```python
from build123d import *

# Parameters (mm, degrees)
SKETCH1_W          = 50
SKETCH1_H          = 70
M16_TAPPED_HOLE1_D = 14
CIRPATTERN1_COUNT  = 4


with BuildPart() as part:
    # Sketch1 → Revolve1 (revolve)
    with BuildSketch(Plane.XY, mode=Mode.PRIVATE) as revolve1_sk:
        with Locations((0, 65)):
            Rectangle(SKETCH1_W, SKETCH1_H)
    revolve(revolve1_sk.sketch.rotate(Axis((71.901236476, 0, 0), (-1, 0, 0)), 90), axis=Axis((71.901236476, 0, 0), (-1, 0, 0)))

    # M16 Tapped Hole1 (through all)
    with Locations(Plane(origin=(-25, 0, -75), x_dir=(0, 0, -1), z_dir=(-1, 0, 0))):
        with Locations((0, 0)):
            m16_tapped_hole1 = Hole(M16_TAPPED_HOLE1_D / 2)

    # CirPattern1: M16 Tapped Hole1 ×4 about axis
    cirpattern1_axis = Axis((0, 0, 0), (1, 0, 0))
    for i in range(1, CIRPATTERN1_COUNT):
        add(m16_tapped_hole1.rotate(cirpattern1_axis, i * 360 / CIRPATTERN1_COUNT), mode=Mode.SUBTRACT)


solid = part.part
```
Can you work these out from the model? Positions are in its coordinate system, mm. Give positions to 0.01 mm unless a question says otherwise; leave off trailing zeros. Order: outer loops, then holes, each group sorted by start corner. A loop starts at its lowest first (then second) coordinate and runs counter-clockwise, first axis right, second up. Notation, with made-up numbers: M 87,70 L 122,70 A13 ccw 122,93 Z; hole C 17,-35.75 d1. An arc over 180 degrees is marked long. Write item = value, one per line. Start each with the question number.
Q1. Suppose I cut it at C-C (x = -4.5). Write out the boundary of the cut face in (y, z).
Q2. Suppose I cut it at A-A (y = 0). Write out the boundary of the cut face in (x, z).
Q3. Suppose I cut it at D-D (y = -75). Write out the boundary of the cut face in (x, z).
Q4. We'd pull the mould along Z, two halves only. Please class faces 1 (the flat face through (25, 21, -24)), 2 (the cylindrical face through (0, 0, -82)), 3 (the cylindrical face through (0.35, -30.04, -95.38)): pulls with the +Z half, pulls with the -Z half, needs draft (parallel to the pull), parting line crosses it, or undercut.
Q5. I need wall thicknesses on probe 1 along Z at (x, y) = (2.5, 3.5); probe 2 along Y at (x, z) = (21, -69); probe 3 along Y at (x, z) = (11.5, -75). Which ranges of each line are inside material? Lowest first, please. Write a range as [from, to].
Q6. Will these pins go through, and if not, where does the flat tip stop? pin 1 Ø18 at (y, z) = (0, -75) entering from +X; pin 2 Ø4 at (x, y) = (0.5, 33) entering from +Z; pin 3 Ø10 at (x, y) = (9.5, -8.5) entering from -Z; pin 4 Ø1.5 at (x, y) = (16.5, 35.5) entering from -Z.
Q7. Suppose I cut it at B-B (z = -25.5). Write out the boundary of the cut face in (x, y).
Check result:
q1.outline = C 0,0 d200; hole C -75,0 d14; hole C 0,0 d60; hole C 0,-75 d14; hole C 0,75 d14; hole C 75,0 d14
q2.outline = M -25,-100 L 25,-100 L 25,-82 L -25,-82 Z; M -25,-68 L 25,-68 L 25,-30 L -25,-30 Z; M -25,30 L 25,30 L 25,68 L -25,68 Z; M -25,82 L 25,82 L 25,100 L -25,100 Z
q3.outline = M -25,-66.14 L 25,-66.14 L 25,-7 L -25,-7 Z; M -25,7 L 25,7 L 25,66.14 L -25,66.14 Z
q4.face_1 = needs draft
q4.face_2 = undercut
q4.face_3 = parting line crosses it
q5.probe_1 = [-99.94, -81.06], [-68.94, -29.8], [29.8, 68.94], [81.06, 99.94]
q5.probe_2 = [-72.38, -3.61], [3.61, 72.38]
q5.probe_3 = [-66.14, -7], [7, 66.14]
q6.pin_1 = 25
q6.pin_2 = 95.07
q6.pin_3 = -99.94
q6.pin_4 = -93.77
q7.outline = M -25,-96.69 L 25,-96.69 L 25,-15.8 L -25,-15.8 Z; M -25,15.8 L 25,15.8 L 25,96.69 L -25,96.69 Z
